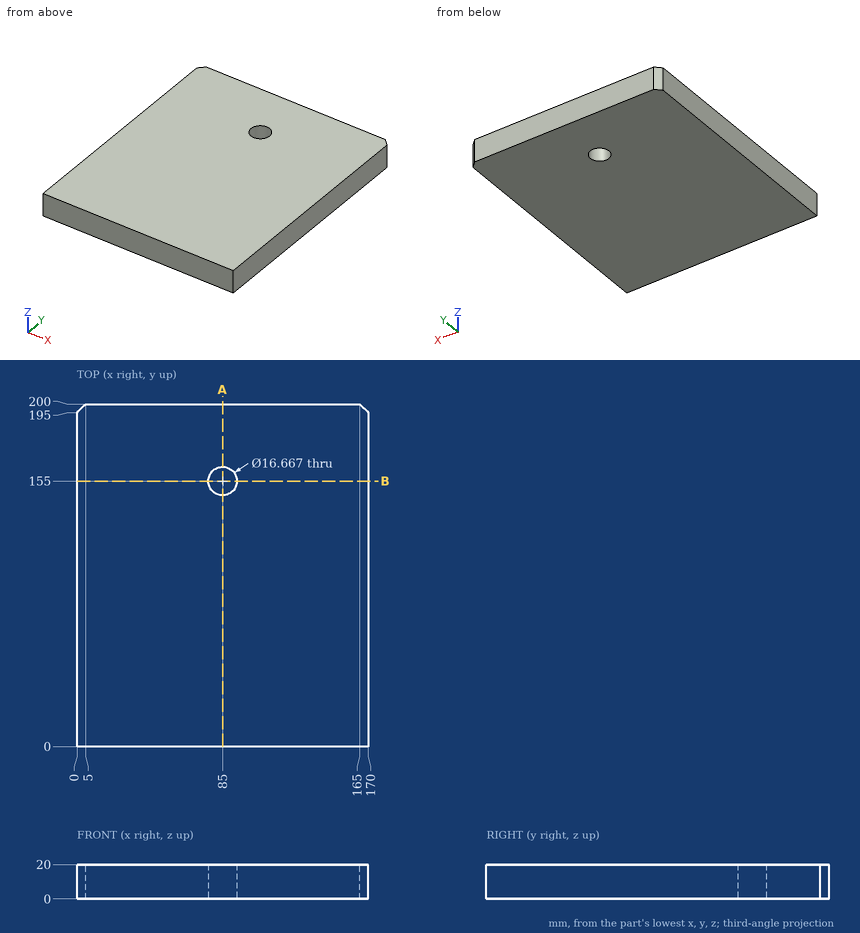
Design review of the part shown in the three views and the two pictorial views. Dimensions are in mm from the part's minimum x, y and z. Round coordinates to 2 decimals unless told otherwise and drop trailing zeros. Loops run counter-clockwise (first coordinate to the right, second up) from the corner with the lowest first, then second, coordinate; pieces in that order, holes last. Notation, with made-up numbers: M 61.25,35 L 70.25,35 A5 cw 70.25,44 Z; hole C -6.5,71.5 d11. An arc over 180 degrees is marked long. Answer as a JSON object with one key per item and string values.
Item 1: Clearance check with a flat-ended pin moving along its axis: P1, Ø12, axis at y = 66.5, z = 2.5, coming from the -X side. State where the tip first meets the part, or that it passes through.
Check sheet entries:
{"P1": "x = 0"}
Item 2: We need section A-A, the plane x = 85. State the section outline as (y, z) points.
Check sheet entries:
{"outline": "M 0,0 L 146.67,0 L 146.67,20 L 0,20 Z; M 163.33,0 L 200,0 L 200,20 L 163.33,20 Z"}
Item 3: We need section B-B, the plane y = 155. State the section outline as (x, z) points.
Check sheet entries:
{"outline": "M 0,0 L 76.67,0 L 76.67,20 L 0,20 Z; M 93.33,0 L 170,0 L 170,20 L 93.33,20 Z"}
Item 4: For line 1 along Y through (x, z) = (85, 8.25); line 2 along X through (y, z) = (159.5, 6.25) (1 decimal); line 3 along Y through (x, z) = (80.5, 4) (1 decimal), list the stretches that pass through material, from the lowest coordinate up.
Check sheet entries:
{"line 1": "0 to 146.67, 163.33 to 200", "line 2": "0 to 78, 92 to 170", "line 3": "0 to 148, 162 to 200"}
